Part model, mm, in its own coordinate system. A direction names the side the tool comes from. Coordinates: 2 decimals unless noted, no trailing zeros. Loops run counter-clockwise (first coordinate to the right, second up) from the corner with the lowest first, then second, coordinate; pieces in that order, holes last. Notation, with made-up numbers: (46, 49) - (89, 49) arc R21 cw to (89, 65) - close; hole circle Ø4 at (48, 24). An arc over 180 degrees is marked (long way). Use a Markdown table: item, result. Add a question column.
1. 3-axis set-ups, long thin cutter, end or side, ignore diameter. For faces 1 (the flat face through (4, 24, 685)), 2 (the flat face through (0, 20, 685)): which of +Z, -Z, +X, -X, +Y, -Y reach the whole face in a straight line?
2. Band-saw the part on A-A, the plane z = 166. Give the cut face in (x, y), plus the area to 3 significant figures.
3. Band-saw the part on B-B, the plane y = 32. Give the cut face in (x, z), plus the area to 3 significant figures.
4. Drop flat-ended pins along their axis: pin 1 (6 mm diameter, centred on x = 26, z = 600.5, fed in from -Y); pin 2 (4 mm diameter, centred on x = 12, z = 759, fed in from +Y); pin 3 (2 mm diameter, centred on x = 7, z = 672.5, fed in from +Y); pin 4 (9 mm diameter, centred on y = 17, z = 514, fed in from +X). Give the stop position or say it passes through.
5. Wall check: probe 1 along Y at (x, z) = (27.5, 798.5); probe 2 along Y at (x, z) = (8, 863). Give the ranges that are in metal, low to high. Write a range as [from, to].
from build123d import *

# Parameters (mm, degrees)
BOSS_EXTRUDE1_DEPTH = 1389


with BuildPart() as part:
    # Sketch1 → Boss-Extrude1 (new body)
    with BuildSketch(Plane.XY):
        with BuildLine():
            Line((0, 0), (0, 40))
            Line((0, 40), (2.666666667, 40))
            ThreePointArc((2.666666667, 40), (3.609475708, 39.609475708), (4, 38.666666667))
            Line((4, 38.666666667), (4, 9))
            ThreePointArc((4, 9), (5.464466094, 5.464466094), (9, 4))
            Line((9, 4), (38.666666667, 4))
            ThreePointArc((38.666666667, 4), (39.609475708, 3.609475708), (40, 2.666666667))
            Line((40, 2.666666667), (40, 0))
            Line((40, 0), (0, 0))
        make_face()
    extrude(amount=BOSS_EXTRUDE1_DEPTH)


solid = part.part
Geometry check:
| question | item | result |
|---|---|---|
| 1 | face 1 | +Z, -Z, +X, +Y |
| 1 | face 2 | +Z, -Z, -X, +Y, -Y |
| 2 | outline | (0, 0) - (40, 0) - (40, 2.67) arc R1.33 ccw to (38.67, 4) - (9, 4) arc R5 cw to (4, 9) - (4, 38.67) arc R1.33 ccw to (2.67, 40) - (0, 40) - close |
| 2 | area | 309 mm^2 |
| 3 | outline | (0, 0) - (4, 0) - (4, 1389) - (0, 1389) - close |
| 3 | area | 5,560 mm^2 |
| 4 | pin 1 | stops at y = 0 |
| 4 | pin 2 | stops at y = 4 |
| 4 | pin 3 | stops at y = 5 |
| 4 | pin 4 | stops at x = 4 |
| 5 | probe 1 | y = [0, 4] |
| 5 | probe 2 | y = [0, 4.1] |
